The model under review builds one solid part; all positions refer to its coordinate system, in mm. A direction names the side the tool comes from. Round coordinates to 2 decimals unless told otherwise and drop trailing zeros. Write each loop counter-clockwise with the first axis right and the second up, starting at its lowest first coordinate (ties: lowest second). Pieces come first, ordered by that corner, then holes. Notation, with made-up numbers: (33, -23.75) -> (83, -23.75) arc R29 cw to (83, 13.25) -> close; hole circle Ø5 at (14, 41). An arc over 180 degrees is marked (long way). Answer as a JSON object with one key per item and string values. Group by question number.
1) We need section B-B, the plane y = 28. Write out the cut boundary in (x, z), then the cut area to 3 significant figures.
2) Machinability: for faces 4 (the flat face through (-1, 30, 21)), 5 (the flat face through (34, 12, -5)), 6 (the cylindrical face through (-30, 26, 0)), which of the approach directions +Z, -Z, +X, -X, +Y, -Y give a long, thin tool a straight path to every point of the face, cutting with its end or side? Answer none if there is none.
3) Mouldability with a two-part tool opening along Y and no side actions: class faces 1 (the cylindrical face through (-7.14, 22.48, -21.46)), 2 (the flat face through (18, 14, 0)), 3 (the flat face through (-1, 30, -22)) as pulls with the +Y half, pulls with the -Y half, needs draft (parallel to the pull), parting line crosses it, or undercut.
4) Insertion check: pin 1 Ø5.5 at (x, z) = (-6, -22.5) entering from +Y; pin 2 Ø1 at (x, z) = (-20, 9.5) entering from +Y; pin 3 Ø14.5 at (x, y) = (0, 17) entering from -Z; pin 4 Ø11 at (x, z) = (30, 3.5) entering from +Y. Each pin has a flat end and moves straight along its axis. Give the tip position at first contact, or say it passes through.
5) We need section A-A, the plane x = 36. Write out the cut boundary in (y, z).
6) We need section C-C, the plane x = 0. Write out the cut boundary in (y, z).
7) To check wall thickness, follow probe 1 along Z at (x, y) = (22.5, 10.5); probe 2 along X at (y, z) = (17, -21.8); probe 3 along Y at (x, z) = (0, 21.5). State the ranges of each line that lie inside material, in increasing order. Write a range as [from, to].
8) We need section D-D, the plane y = 17. Write out the cut boundary in (x, z).
from build123d import *

# Parameters (mm, degrees)
BASE_BLOCK_SKETCH_W         = 90
BASE_BLOCK_SKETCH_H         = 48
BASE_BLOCK_90X48X30_DEPTH   = 30
CHANNEL_SKETCH_W            = 38
CHANNEL_SKETCH_H            = 25
U_CHANNEL_CUT_DEPTH         = 98.857038582
HALF_CYLINDER_POST_30_DEPTH = 48
POST_BORE_SKETCH_R          = 9
POST_BORE_18_DEPTH          = 48
END_TAB_SKETCH_W            = 27
END_TAB_SKETCH_H            = 22
END_TAB_DEPTH               = 19
END_TAB_SLOT_SKETCH_W       = 21
END_TAB_SLOT_SKETCH_H       = 10
END_TAB_SLOT_DEPTH          = 57.364882684
SIDE_HOLE_SKETCH_R          = 9
SIDE_HOLE_18_DEPTH          = 19
OPPOSITE_START              = -19
OPPOSITE_SIDE_HOLE_SKETCH_R = 9
OPPOSITE_SIDE_HOLE_18_DEPTH = 19


with BuildPart() as part:
    # Base Block Sketch → Base Block 90x48x30 (new body)
    with BuildSketch(Plane(origin=(0, 0, 0), x_dir=(1, 0, 0), z_dir=(0, 1, 0))):
        Rectangle(BASE_BLOCK_SKETCH_W, BASE_BLOCK_SKETCH_H)
    extrude(amount=BASE_BLOCK_90X48X30_DEPTH)

    # Channel Sketch → U-Channel Cut (cut, through all)
    with BuildSketch(Plane.ZY.offset(45)):
        with Locations((0, 17.5)):
            Rectangle(CHANNEL_SKETCH_W, CHANNEL_SKETCH_H)
    extrude(amount=-U_CHANNEL_CUT_DEPTH, mode=Mode.SUBTRACT)

    # Half Cylinder Post Sketch → Half Cylinder Post Ø30 (add)
    with BuildSketch(Plane.XZ):
        with BuildLine():
            Line((-45, 15), (-45, -15))
            ThreePointArc((-45, -15), (-30, 0), (-45, 15))
        make_face()
    extrude(amount=-HALF_CYLINDER_POST_30_DEPTH)

    # Post Bore Sketch → Post Bore Ø18 (cut)
    with BuildSketch(Plane(origin=(0, 48, 0), x_dir=(1, 0, 0), z_dir=(0, 1, 0))):
        with Locations((-45, 0)):
            Circle(POST_BORE_SKETCH_R)
    extrude(amount=-POST_BORE_18_DEPTH, mode=Mode.SUBTRACT)

    # End Tab Sketch → End Tab (add)
    with BuildSketch(Plane(origin=(0, 5, 0), x_dir=(1, 0, 0), z_dir=(0, 1, 0))):
        with Locations((31.5, 0)):
            Rectangle(END_TAB_SKETCH_W, END_TAB_SKETCH_H)
    extrude(amount=END_TAB_DEPTH)

    # End Tab Slot Sketch → End Tab Slot (cut, through all)
    with BuildSketch(Plane(origin=(0, 24, 0), x_dir=(1, 0, 0), z_dir=(0, 1, 0))):
        with Locations((34.5, 0)):
            Rectangle(END_TAB_SLOT_SKETCH_W, END_TAB_SLOT_SKETCH_H)
    extrude(amount=-END_TAB_SLOT_DEPTH, mode=Mode.SUBTRACT)

    # Side Hole Sketch → Side Hole Ø18 (cut)
    with BuildSketch(Plane.XY.offset(24)):
        with Locations((0, 17)):
            Circle(SIDE_HOLE_SKETCH_R)
    extrude(amount=-SIDE_HOLE_18_DEPTH, mode=Mode.SUBTRACT)

    # Opposite Side Hole Sketch → Opposite Side Hole Ø18 (cut)
    with BuildSketch(Plane(origin=(0, 0, -24), x_dir=(-1, 0, 0), z_dir=(0, 0, -1)).offset(OPPOSITE_START)):
        with Locations(Location((0, 17, 0), (0, 0, 180))):
            Circle(OPPOSITE_SIDE_HOLE_SKETCH_R)
    extrude(amount=OPPOSITE_SIDE_HOLE_18_DEPTH, mode=Mode.SUBTRACT)


solid = part.part
Here are the results:
{
 "1": {"outline": "(-45, -24) -> (45, -24) -> (45, -19) -> (-45, -19) -> close; (-45, -15) arc R15 ccw to (-45, 15) -> (-45, 9) arc R9 cw to (-45, -9) -> close; (-45, 19) -> (45, 19) -> (45, 24) -> (-45, 24) -> close", "area": "1,130 mm^2"},
 "2": {"face 4": "+Z, +X, -X, +Y", "face 5": "+X, +Y, -Y", "face 6": "+Y"},
 "3": {"face 1": "undercut", "face 2": "needs draft", "face 3": "pulls with the +Y half"},
 "4": {"pin 1": "stops at y = 30", "pin 2": "stops at y = 5", "pin 3": "passes through", "pin 4": "stops at y = 24"},
 "5": {"outline": "(0, -24) -> (30, -24) -> (30, -19) -> (5, -19) -> (5, -11) -> (24, -11) -> (24, -5) -> (0, -5) -> close; (0, 5) -> (24, 5) -> (24, 11) -> (5, 11) -> (5, 19) -> (30, 19) -> (30, 24) -> (0, 24) -> close"},
 "6": {"outline": "(0, -24) -> (8, -24) -> (8, -19) -> (5, -19) -> (5, 19) -> (8, 19) -> (8, 24) -> (0, 24) -> close; (26, -24) -> (30, -24) -> (30, -19) -> (26, -19) -> close; (26, 19) -> (30, 19) -> (30, 24) -> (26, 24) -> close"},
 "7": {"probe 1": "z = [-24, -19], [-11, 11], [19, 24]", "probe 2": "x = [-45, -9], [9, 45]", "probe 3": "y = [0, 8], [26, 30]"},
 "8": {"outline": "(-45, -24) -> (-9, -24) -> (-9, -19) -> (-45, -19) -> close; (-45, -15) arc R15 ccw to (-45, 15) -> (-45, 9) arc R9 cw to (-45, -9) -> close; (-45, 19) -> (-9, 19) -> (-9, 24) -> (-45, 24) -> close; (9, -24) -> (45, -24) -> (45, -19) -> (9, -19) -> close; (9, 19) -> (45, 19) -> (45, 24) -> (9, 24) -> close; (18, -11) -> (45, -11) -> (45, -5) -> (24, -5) -> (24, 5) -> (45, 5) -> (45, 11) -> (18, 11) -> close"}
}
